```python
from build123d import *

# Parameters (mm, degrees)
SKETCH1_R           = 100
BOSS_EXTRUDE1_DEPTH = 100


with BuildPart() as part:
    # Sketch1 → Boss-Extrude1 (new body)
    with BuildSketch(Plane.XY):
        Polygon((200, 50), (2050, 50), (2050, 200), (2450, 200), (2450, -200), (2050, -200), (2050, -50), (200, -50), (200, -200), (-200, -200), (-200, 200), (200, 200), align=None)
        Circle(SKETCH1_R, mode=Mode.SUBTRACT)
        with Locations((2250, 0)):
            Circle(SKETCH1_R, mode=Mode.SUBTRACT)
    extrude(amount=BOSS_EXTRUDE1_DEPTH)


solid = part.part
```
The listing builds one solid part. Answer for the finished solid, in the listing's coordinates (mm). A direction names the side the tool comes from. Round coordinates to 2 decimals unless told otherwise and drop trailing zeros. Order: outer loops, then holes, each group sorted by start corner. A loop starts at its lowest first (then second) coordinate and runs counter-clockwise, first axis right, second up. Notation, with made-up numbers: (17, -3.75) -> (39, -3.75) arc R35 ccw to (39, 28.25) -> close; hole circle Ø4 at (41.25, -22). An arc over 180 degrees is marked (long way). Answer as CSV lines item,"result". Start each with the question number.
(1) The part is cut by section C-C (x = 0). Determine the outline of the cut face in (y, z), then the cut area to 3 significant figures.
(2) A tool of negligible diameter and unlimited length cuts with its end or side. For faces 1 (the face through (1138, -50, 49)), 2 (the face through (3, -200, 49)), 3 (the face through (200, 126, 49)), from which of +Z, -Z, +X, -X, +Y, -Y can it reach the whole face along a straight path? Write none if from no direction.
(3) Flat-ended cylindrical pins translate along their axes: pin 1 Ø10 at (x, z) = (397, 75) entering from -Y; pin 2 Ø6 at (x, z) = (1200.5, 68.5) entering from +Y. Find the tip coordinate at first contact, or state that the pin passes through.
(4) Find the intervals of material crossed by probe 1 along Y at (x, z) = (0, 78); probe 2 along X at (y, z) = (77, 44); probe 3 along X at (y, z) = (137.5, 5.5), in increasing order. Write a range as from..to.
(5) The part is cut by section A-A (y = 0). Determine the outline of the cut face in (x, z).
(6) The part is cut by section D-D (y = -163). Determine the outline of the cut face in (x, z), then the cut area to 3 significant figures.
(7) The part is cut by section B-B (z = 36). Determine the outline of the cut face in (x, y).
(8) For a pull along X with two mould halves and no side action, classify faces 4 (the face through (-200, -3, 49)), 5 (the face through (200, -124, 49)), 6 (the face through (2450, 3, 49)), 7 (the face through (1144, 3, 100)) as +X half, -X half, draft (parallel to the pull), parting line (faces both ways), or undercut.
Evaluation:
1,outline,"(-200, 0) -> (-100, 0) -> (-100, 100) -> (-200, 100) -> close; (100, 0) -> (200, 0) -> (200, 100) -> (100, 100) -> close"
1,area,"20,000 mm²"
2,face 1,"+Z, -Z, -Y"
2,face 2,"+Z, -Z, +X, -X, -Y"
2,face 3,"+Z, -Z, +Y"
3,pin 1,"y = -50"
3,pin 2,"y = 50"
4,probe 1,"-200..-100, 100..200"
4,probe 2,"-200..-63.8, 63.8..200, 2050..2186.2, 2313.8..2450"
4,probe 3,"-200..200, 2050..2450"
5,outline,"(-200, 0) -> (-100, 0) -> (-100, 100) -> (-200, 100) -> close; (100, 0) -> (2150, 0) -> (2150, 100) -> (100, 100) -> close; (2350, 0) -> (2450, 0) -> (2450, 100) -> (2350, 100) -> close"
6,outline,"(-200, 0) -> (200, 0) -> (200, 100) -> (-200, 100) -> close; (2050, 0) -> (2450, 0) -> (2450, 100) -> (2050, 100) -> close"
6,area,"80,000 mm²"
7,outline,"(-200, -200) -> (200, -200) -> (200, -50) -> (2050, -50) -> (2050, -200) -> (2450, -200) -> (2450, 200) -> (2050, 200) -> (2050, 50) -> (200, 50) -> (200, 200) -> (-200, 200) -> close; hole circle Ø200 at (0, 0); hole circle Ø200 at (2250, 0)"
8,face 4,"-X half"
8,face 5,"undercut"
8,face 6,"+X half"
8,face 7,"draft"
